```python
from build123d import *

# Parameters (mm, degrees)
SKETCH1_W             = 75
SKETCH1_H             = 14
BOSS_EXTRUDE1_DEPTH   = 200
SKETCH2_R             = 17.5
CUT_EXTRUDE1_DEPTH    = 226.39507559
M8_TAPPED_HOLE2_D     = 6.8
M8_TAPPED_HOLE2_DEPTH = 22.25
M8_TAPPED_HOLE2_TIP   = 2.042926105
M8_TAPPED_HOLE3_D     = 6.8
M8_TAPPED_HOLE3_DEPTH = 22.25
M8_TAPPED_HOLE3_TIP   = 2.042926105


with BuildPart() as part:
    # Sketch1 → Boss-Extrude1 (new body)
    with BuildSketch(Plane.XY):
        with Locations((65.49, 327)):
            Rectangle(SKETCH1_W, SKETCH1_H)
    extrude(amount=BOSS_EXTRUDE1_DEPTH)

    # Sketch2 → Cut-Extrude1 (cut, through all)
    with BuildSketch(Plane(origin=(0, 334, 0), x_dir=(1, 0, 0), z_dir=(0, 1, 0))):
        with Locations(Location((65.49, -100, 0), (0, 0, 270))):
            Circle(SKETCH2_R)
    extrude(amount=-CUT_EXTRUDE1_DEPTH, mode=Mode.SUBTRACT)

    # M8 Tapped Hole2
    with Locations(Plane.XY.offset(200)):
        with Locations((65.49, 327), (40.49, 327), (90.49, 327)):
            Hole(M8_TAPPED_HOLE2_D / 2, depth=M8_TAPPED_HOLE2_DEPTH)
            with Locations((0, 0, -(M8_TAPPED_HOLE2_DEPTH + M8_TAPPED_HOLE2_TIP / 2))):  # 118° drill point
                Cone(0, M8_TAPPED_HOLE2_D / 2, M8_TAPPED_HOLE2_TIP, mode=Mode.SUBTRACT)

    # M8 Tapped Hole3
    with Locations(Plane(origin=(0, 0, 0), x_dir=(-1, 0, 0), z_dir=(0, 0, -1))):
        with Locations((-90.49, 327), (-65.49, 327), (-40.49, 327)):
            Hole(M8_TAPPED_HOLE3_D / 2, depth=M8_TAPPED_HOLE3_DEPTH)
            with Locations((0, 0, -(M8_TAPPED_HOLE3_DEPTH + M8_TAPPED_HOLE3_TIP / 2))):  # 118° drill point
                Cone(0, M8_TAPPED_HOLE3_D / 2, M8_TAPPED_HOLE3_TIP, mode=Mode.SUBTRACT)


solid = part.part
```
Work out the finished part from the listing and answer in its coordinate system (mm). A direction names the side the tool comes from. Round coordinates to 2 decimals unless told otherwise and drop trailing zeros. Loops run counter-clockwise (first coordinate to the right, second up) from the corner with the lowest first, then second, coordinate; pieces in that order, holes last. Notation, with made-up numbers: M 54,61.25 L 100,61.25 A20 cw 100,90.25 Z; hole C 37,67.25 d3. An arc over 180 degrees is marked long. One line per question, with ' | ' between items.
Q1. Find section A-A, the plane z = 100. Give the vertices of the cut face in (x, y).
Conclusion:
outline: M 27.99,320 L 47.99,320 L 47.99,334 L 27.99,334 Z; M 82.99,320 L 102.99,320 L 102.99,334 L 82.99,334 Z
Q2. The mould has two halves that part along X. Classify faces 1 (the flat face through (102.99, 327, 99)), 2 (the flat face through (65, 334, 76)), 3 (the conical face through (65.807, 327.498, 176.062)): +X half, -X half, draft (parallel to the pull), parting line (faces both ways), or undercut.
Conclusion:
face 1: +X half | face 2: draft | face 3: undercut
Q3. Each of these flat-tipped pins is pushed along its axis until it touches: pin 1 Ø5.5 at (x, y) = (40.49, 327) entering from -Z; pin 2 Ø6 at (x, y) = (40.49, 327) entering from -Z; pin 3 Ø4 at (x, y) = (90.49, 327) entering from +Z. Where does it stop, or does it pass through?
Conclusion:
pin 1: stops at z = 22.64 | pin 2: stops at z = 22.49 | pin 3: stops at z = 176.91
Q4. A tool of negligible diameter and unlimited length cuts with its end or side. For faces 4 (the flat face through (65, 322, 200)), 5 (the cylindrical face through (39.75, 323.68, 11.28)), 6 (the cylindrical face through (87.35, 325.7, 188.72)), from which of +Z, -Z, +X, -X, +Y, -Y can it reach the whole face along a straight path? Write none if from no direction.
Conclusion:
face 4: +Z, +X, -X, +Y, -Y | face 5: -Z | face 6: +Z
Q5. Consider line 1 along X through (y, z) = (327, 193.25); line 2 along Y through (x, z) = (65.49, 183.5); line 3 along Z through (x, y) = (66.5, 331.5). Determine where each line is inside the solid, lowest interval first. Write a range as from..to.
Conclusion:
line 1: x = 27.99..37.09, 43.89..62.09, 68.89..87.09, 93.89..102.99 | line 2: y = 320..323.6, 330.4..334 | line 3: z = 0..82.53, 117.47..200
